Model file for the job. Use its own axes, mm. Face numbers are marked on the shaded views. A direction names the side the tool comes from. Round coordinates to 2 decimals unless told otherwise and drop trailing zeros. Order: outer loops, then holes, each group sorted by start corner. A loop starts at its lowest first (then second) coordinate and runs counter-clockwise, first axis right, second up. Notation, with made-up numbers: (14, -3) -> (66, -3) arc R19 ccw to (66, 30) -> close; hole circle Ø6 at (39, 0.25). An arc over 180 degrees is marked (long way). Answer as CSV lines item,"result".
```python
from build123d import *

# Parameters (mm, degrees)
BRACKET_BODY_DEPTH            = 125
PLATE_RELIEF_CUT_DEPTH        = 36
CROSS_HOLES_CUT_11_DEEP_DEPTH = 11
SKETCH3_4_R                   = 6.5
CROSS_HOLES_CUT_36_DEEP_DEPTH = 36
HOLE_12_SKETCH_R              = 6
HOLE_12_DEPTH                 = 11


with BuildPart() as part:
    # Bracket Profile Sketch → Bracket Body (new body)
    with BuildSketch(Plane.XY):
        Polygon((-36, 0), (0, 0), (0, 16), (0, 17.641196013), (0, 90), (-36, 90), align=None)
        Polygon((0, 0), (32, 0), (32, 4), (17.698956889, 16), (0, 16), align=None)
    extrude(amount=BRACKET_BODY_DEPTH)

    # Plate Relief Sketch → Plate Relief Cut (cut)
    with BuildSketch(Plane.ZY.offset(36)):
        Polygon((12, 90), (111.955126335, 0), (125, 0), (125, 90), align=None)
    extrude(amount=-PLATE_RELIEF_CUT_DEPTH, mode=Mode.SUBTRACT)

    # Cross Holes Sketch → Cross Holes Cut 11 Deep (cut)
    with BuildSketch(Plane.ZY.offset(36)):
        Polygon((-5.668578971, 51.118217594), (-13.477683521, 103.633494759), (27.976080454, 91.378914898), (26.142244571, 82.929041136), align=None)
    extrude(amount=-CROSS_HOLES_CUT_11_DEEP_DEPTH, mode=Mode.SUBTRACT)

    # Sketch3_4 → Cross Holes Cut 36 Deep (cut)
    with BuildSketch(Plane.ZY.offset(36)):
        with Locations((19.871294507, 56)):
            Circle(SKETCH3_4_R)
        with Locations((47.636607378, 31)):
            Circle(SKETCH3_4_R)
    extrude(amount=-CROSS_HOLES_CUT_36_DEEP_DEPTH, mode=Mode.SUBTRACT)

    # Hole _12 Sketch → Hole _12 (cut)
    with BuildSketch(Plane(origin=(0, 55.670912219, 50.126314512), x_dir=(1, 0, 0), z_dir=(0, 0.7431448254773981, 0.669130606358854))):
        with Locations(Location((-16, -16.198872821, 0), (0, 0, 270))):
            Circle(HOLE_12_SKETCH_R)
    extrude(amount=-HOLE_12_DEPTH, mode=Mode.SUBTRACT)


solid = part.part
```
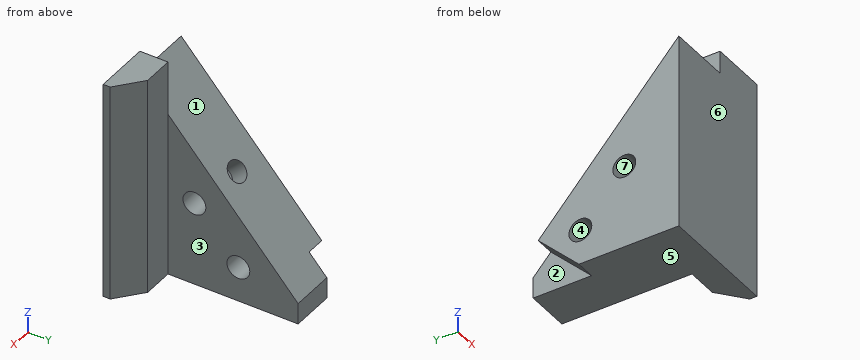
Q1. Saw through at D-D (z = 45). Write the cut outline in (x, y), plus the area to 3 significant figures.
Checks:
outline,"(-36, 0) -> (32, 0) -> (32, 4) -> (17.7, 16) -> (0, 16) -> (0, 25.06) -> (-36, 25.06) -> close; (-36, 36.94) -> (0, 36.94) -> (0, 60.29) -> (-36, 60.29) -> close"
area,"2,170 mm²"
Q2. Saw through at A-A (y = 31). Write the cut outline in (x, z), plus the area to 3 significant figures.
Checks:
outline,"(-36, 0) -> (0, 0) -> (0, 41.14) -> (-36, 41.14) -> close; (-36, 54.14) -> (0, 54.14) -> (0, 77.53) -> (-36, 77.53) -> close"
area,"2,320 mm²"
Q3. Wall check: L1, parallel to Y at x = 11.5, z = 120; L2, parallel to Y at x = -14, z = 56.5; L3, parallel to Z at x = -3, y = 27. Give the ranges that are in metal, low to high. Write a range as [from, to].
Checks:
L1,"[0, 16]"
L2,"[0, 35.13], [46.99, 49.93]"
L3,"[0, 42.51], [52.76, 81.97]"
Q4. Mould opens along Z. For the marked faces 4, 5, 6 and 7 say: +Z half, -Z half, draft (parallel to the pull), parting line (faces both ways), or undercut.
Checks:
face 4,"undercut"
face 5,"-Z half"
face 6,"draft"
face 7,"undercut"
Q5. Saw through at B-B (z = 28). Write the cut outline in (x, y), plus the area to 3 significant figures.
Checks:
outline,"(-36, 0) -> (32, 0) -> (32, 4) -> (17.7, 16) -> (0, 16) -> (0, 75.59) -> (-36, 75.59) -> close"
area,"3,150 mm²"
Q6. Saw through at C-C (x = 14.5). Write the cut outline in (y, z).
Checks:
outline,"(0, 0) -> (16, 0) -> (16, 125) -> (0, 125) -> close"
Q7. Flat gauge pins, fed straight in: pin 1 (4 mm diameter, centred on x = -7.5, z = 31.5, fed in from +Y); pin 2 (8 mm diameter, centred on x = 11, z = 51.5, fed in from +Y); pin 3 (8 mm diameter, centred on y = 56, z = 19.87, fed in from -X); pin 4 (5 mm diameter, centred on x = -16, y = 37.5, fed in from +Z). Where does each tip first touch, or does it go through?
Checks:
pin 1,"y = 74.24"
pin 2,"y = 16"
pin 3,"through"
pin 4,"z = 73.08"
Q8. Tool access for the marked faces 1, 2 and 3: list every direction of +Z, -Z, +X, -X, +Y, -Y with a clear straight run to the whole face (end or side of a thin tool).
Checks:
face 1,"+Z, -X, +Y"
face 2,"-Z, -X, +Y"
face 3,"+Z, -Z, +X, +Y"
